Geometry check sheet. Reference: drawing and pictorial views, mm from the part's lowest x, y, z. Give positions to 0.01 mm unless a question says otherwise; leave off trailing zeros. Write each loop counter-clockwise with the first axis right and the second up, starting at its lowest first coordinate (ties: lowest second). Pieces come first, ordered by that corner, then holes. Notation, with made-up numbers: M 33,17.5 L 77,17.5 A14 cw 77,26.5 Z; hole C 12.5,80 d10. An arc over 180 degrees is marked long. One line per item, written item: value. Start each with the question number.
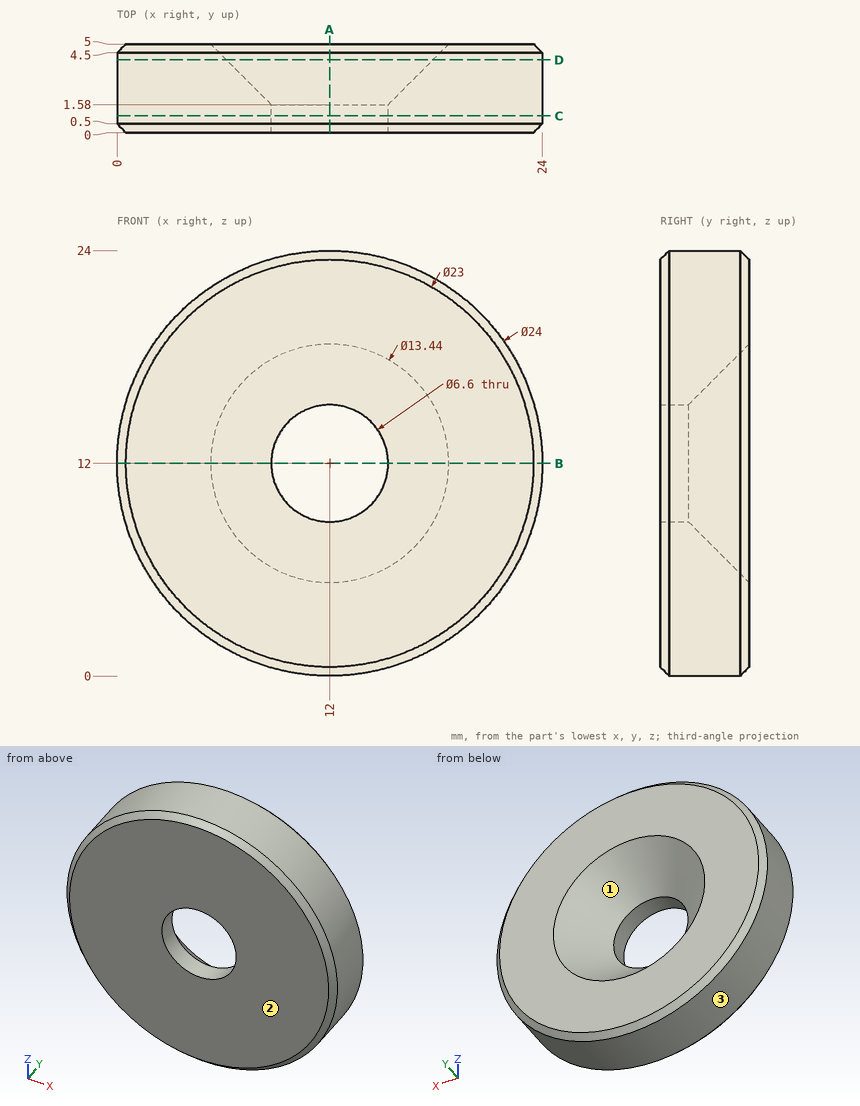
1) Cross-section at B-B (z = 12). Record the boundary of the cut face in (x, y), plus the area to 3 significant figures.
2) Gauge pin test, flat ends, axial feed: pin 1 (2 mm diameter, centred on y = 2, z = 14, fed in from +X); pin 2 (3 mm diameter, centred on x = 5, z = 6.5, fed in from -Y); pin 3 (2 mm diameter, centred on x = 18, y = 4, fed in from +Z); pin 4 (1.5 mm diameter, centred on y = 3, z = 3, fed in from +X). Record the tip position at first contact, or that the pin passes through.
3) Cross-section at C-C (y = 0.95). Record the boundary of the cut face in (x, z).
4) Draft check along Z on the marked faces 1, 2 and 3. Enter one of: released by +Z, released by -Z, zero draft, split by the parting line, or undercut.
5) Cross-section at A-A (x = 12). Record the boundary of the cut face in (y, z), plus the area to 3 significant figures.
6) Cross-section at D-D (y = 4.1). Record the boundary of the cut face in (x, z).
7) Material ranges on L1, parallel to X at y = 0.7, z = 12; L2, parallel to Z at x = 12.75, y = 3.9; L3, parallel to X at y = 3.9, z = 7, recorded low to high. Write a range as from..to.
Data:
1. outline: M 0,0.5 L 0.5,0 L 8.7,0 L 8.7,1.58 L 5.28,5 L 0.5,5 L 0,4.5 Z; M 15.3,0 L 23.5,0 L 24,0.5 L 24,4.5 L 23.5,5 L 18.72,5 L 15.3,1.58 Z
1. area: 74.8 mm2
2. pin 1: stops at x = 23.96
2. pin 2: stops at y = 0
2. pin 3: stops at z = 22.91
2. pin 4: stops at x = 20.71
3. outline: C 12,12 d24; hole C 12,12 d6.6
4. face 1: undercut
4. face 2: zero draft
4. face 3: split by the parting line
5. outline: M 0,0.5 L 0.5,0 L 4.5,0 L 5,0.5 L 5,5.28 L 1.58,8.7 L 0,8.7 Z; M 0,15.3 L 1.58,15.3 L 5,18.72 L 5,23.5 L 4.5,24 L 0.5,24 L 0,23.5 Z
5. area: 74.8 mm2
6. outline: C 12,12 d24; hole C 12,12 d11.64
7. L1: x = 0..8.7, 15.3..24
7. L2: z = 0.02..6.43, 17.57..23.98
7. L3: x = 1.09..9.43, 14.57..22.91
